Check sheet for the drawn part. Datum: minimum x, y, z corner. Units: mm. Coordinates: 2 decimals unless noted, no trailing zeros. Write each loop counter-clockwise with the first axis right and the second up, starting at its lowest first coordinate (ties: lowest second). Pieces come first, ordered by that corner, then holes. Notation, with made-up numbers: M -29.75,-36 L -0.75,-36 A22 cw -0.75,-28 Z; hole C 31.5,35 d11. An arc over 180 degrees is marked long. Answer in a Markdown table with one row per item.
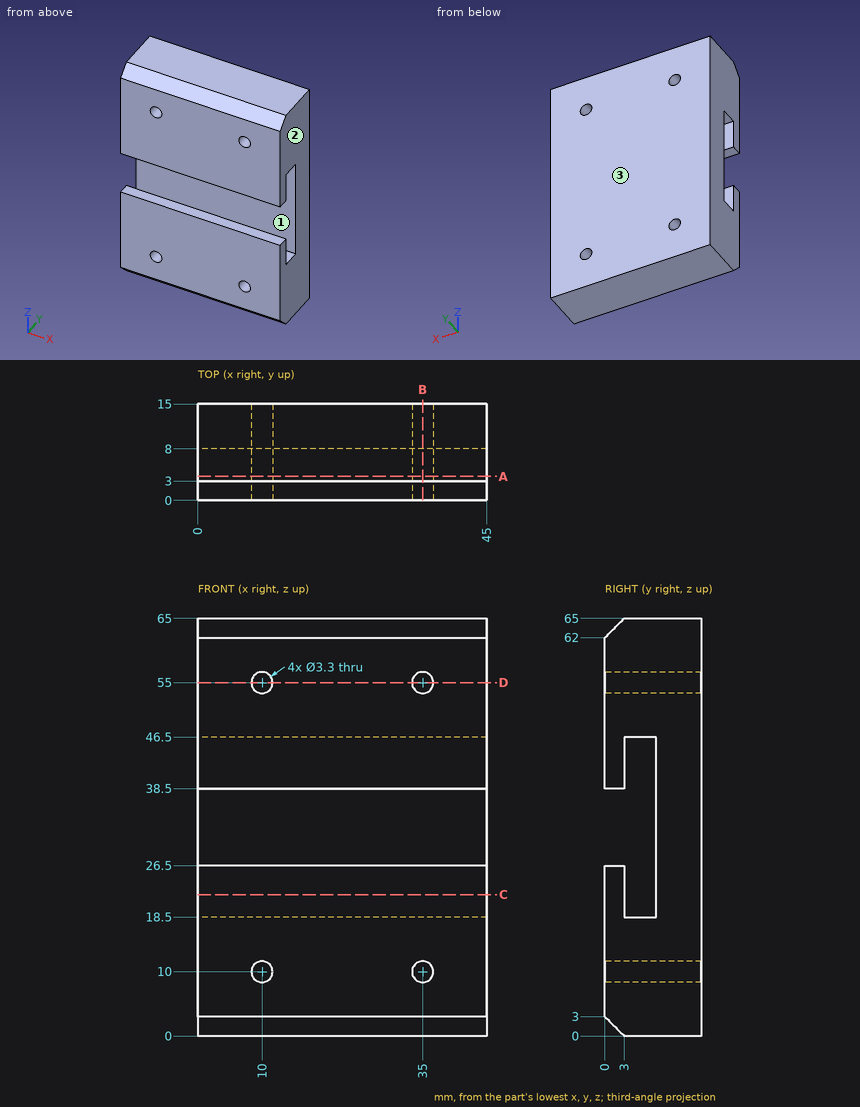
1) Sectioned sample at A-A (y = 3.75). Record the cut outline in (x, z).
Response values:
| item | result |
|---|---|
| outline | M 0,0 L 45,0 L 45,18.5 L 0,18.5 Z; M 0,46.5 L 45,46.5 L 45,65 L 0,65 Z; hole C 10,10 d3.3; hole C 10,55 d3.3; hole C 35,10 d3.3; hole C 35,55 d3.3 |
2) Sectioned sample at B-B (x = 35). Record the cut outline in (y, z), then the cut area to 3 significant figures.
Response values:
| item | result |
|---|---|
| outline | M 0,3 L 3,0 L 15,0 L 15,8.35 L 0,8.35 Z; M 0,11.65 L 15,11.65 L 15,53.35 L 0,53.35 L 0,38.5 L 3,38.5 L 3,46.5 L 8,46.5 L 8,18.5 L 3,18.5 L 3,26.5 L 0,26.5 Z; M 0,56.65 L 15,56.65 L 15,65 L 3,65 L 0,62 Z |
| area | 691 mm² |
3) Thickness scan on L1, parallel to Z at x = 10, y = 4; L2, parallel to X at y = 5.5, z = 10; L3, parallel to Y at x = 30, z = 40. Record the ranges inside material, lowest first. Write a range as [from, to].
Response values:
| item | result |
|---|---|
| L1 | z = [0, 8.35], [11.65, 18.5], [46.5, 53.35], [56.65, 65] |
| L2 | x = [0, 8.35], [11.65, 33.35], [36.65, 45] |
| L3 | y = [0, 3], [8, 15] |
4) Sectioned sample at D-D (z = 55). Record the cut outline in (x, y), then the cut area to 3 significant figures.
Response values:
| item | result |
|---|---|
| outline | M 0,0 L 8.35,0 L 8.35,15 L 0,15 Z; M 11.65,0 L 33.35,0 L 33.35,15 L 11.65,15 Z; M 36.65,0 L 45,0 L 45,15 L 36.65,15 Z |
| area | 576 mm² |
5) Sectioned sample at C-C (z = 22). Record the cut outline in (x, y), then the cut area to 3 significant figures.
Response values:
| item | result |
|---|---|
| outline | M 0,0 L 45,0 L 45,3 L 0,3 Z; M 0,8 L 45,8 L 45,15 L 0,15 Z |
| area | 450 mm² |
6) Release check for a two-part mould opening along Y. For the marked faces 1, 2 and 3 record: +Y half, -Y half, draft (parallel to the pull), parting line (faces both ways), or undercut.
Response values:
| item | result |
|---|---|
| face 1 | undercut |
| face 2 | draft |
| face 3 | +Y half |
7) Depth check by flat-ended pin: pin 1 (2 mm diameter, centred on x = 35, z = 10, fed in from -Y); pin 2 (1.5 mm diameter, centred on x = 15.5, y = 1, fed in from -Z); pin 3 (4 mm diameter, centred on x = 20.5, z = 31, fed in from -Y); pin 4 (3.5 mm diameter, centred on x = 15, y = 1, fed in from +Z). Enter the tip coordinate at first touch or a pass-through.
Response values:
| item | result |
|---|---|
| pin 1 | passes through |
| pin 2 | stops at z = 1.25 |
| pin 3 | stops at y = 8 |
| pin 4 | stops at z = 64.75 |
